Can you work these out from the model? Positions are in its coordinate system, mm. Face numbers are marked on the shaded views. A direction names the side the tool comes from. Round coordinates to 2 decimals unless told otherwise and drop trailing zeros. Order: outer loops, then holes, each group sorted by start corner. A loop starts at its lowest first (then second) coordinate and runs counter-clockwise, first axis right, second up.
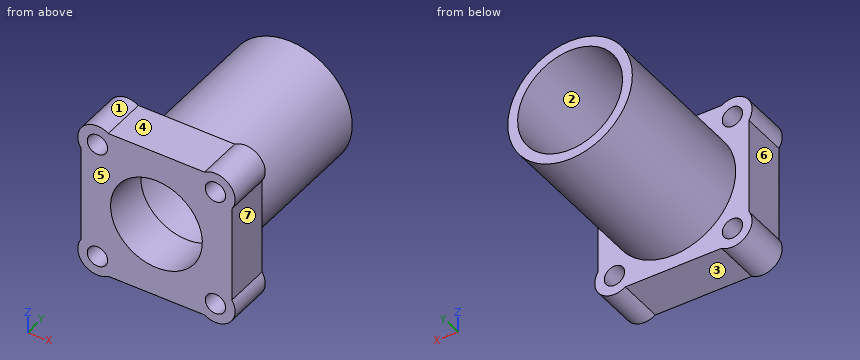
from build123d import *

# Parameters (mm, degrees)
SKETCH_1_R      = 7
SKETCH_1_R_2    = 3
SKETCH_1_R_3    = 1.55
EXTRUDE_1_DEPTH = 7
SKETCH_2_R      = 9.5
SKETCH_2_R_2    = 8
EXTRUDE_2_DEPTH = 24


with BuildPart() as part:
    # 草图1 → 凸台-拉伸1 (new body)
    # profile 1 of 5: a face of its own
    with BuildSketch(Plane(origin=(0, 0, 0), x_dir=(1, 0, 0), z_dir=(0, 1, 0))):
        with BuildLine():
            Line((7.341687605, 11.5), (-7.341687605, 11.5))
            ThreePointArc((-7.341687605, 11.5), (-6.356617963, 10.418637165), (-6, 9))
            ThreePointArc((-6, 9), (-8.133974596, 6.127718677), (-11.5, 7.341687605))
            Line((-11.5, 7.341687605), (-11.5, -7.341687605))
            ThreePointArc((-11.5, -7.341687605), (-8.133974596, -6.127718677), (-6, -9))
            ThreePointArc((-6, -9), (-6.356617963, -10.418637165), (-7.341687605, -11.5))
            Line((-7.341687605, -11.5), (7.341687605, -11.5))
            ThreePointArc((7.341687605, -11.5), (6.878679656, -6.878679656), (11.5, -7.341687605))
            Line((11.5, -7.341687605), (11.5, 7.341687605))
            ThreePointArc((11.5, 7.341687605), (6.878679656, 6.878679656), (7.341687605, 11.5))
        make_face()
        with Locations(Location((0, 0, 0), (0, 0, 270))):
            Circle(SKETCH_1_R, mode=Mode.SUBTRACT)
    # profile 2 of 5: a face of its own
    with BuildSketch(Plane(origin=(0, 0, 0), x_dir=(1, 0, 0), z_dir=(0, 1, 0))):
        with Locations((-9, -9)):
            Circle(SKETCH_1_R_2)
        with Locations(Location((-9, -9, 0), (0, 0, 270))):
            Circle(SKETCH_1_R_3, mode=Mode.SUBTRACT)
    # profile 3 of 5: a face of its own
    with BuildSketch(Plane(origin=(0, 0, 0), x_dir=(1, 0, 0), z_dir=(0, 1, 0))):
        with Locations((9, -9)):
            Circle(SKETCH_1_R_2)
        with Locations(Location((9, -9, 0), (0, 0, 270))):
            Circle(SKETCH_1_R_3, mode=Mode.SUBTRACT)
    # profile 4 of 5: a face of its own
    with BuildSketch(Plane(origin=(0, 0, 0), x_dir=(1, 0, 0), z_dir=(0, 1, 0))):
        with Locations((9, 9)):
            Circle(SKETCH_1_R_2)
        with Locations(Location((9, 9, 0), (0, 0, 270))):
            Circle(SKETCH_1_R_3, mode=Mode.SUBTRACT)
    # profile 5 of 5: a face of its own
    with BuildSketch(Plane(origin=(0, 0, 0), x_dir=(1, 0, 0), z_dir=(0, 1, 0))):
        with Locations((-9, 9)):
            Circle(SKETCH_1_R_2)
        with Locations(Location((-9, 9, 0), (0, 0, 270))):
            Circle(SKETCH_1_R_3, mode=Mode.SUBTRACT)
    extrude(amount=EXTRUDE_1_DEPTH)

    # 草图2 → 凸台-拉伸2 (add)
    with BuildSketch(Plane(origin=(0, 7, 0), x_dir=(1, 0, 0), z_dir=(0, 1, 0))):
        with Locations(Location((0, 0, 0), (0, 0, 270))):
            Circle(SKETCH_2_R)
        with Locations(Location((0, 0, 0), (0, 0, 270))):
            Circle(SKETCH_2_R_2, mode=Mode.SUBTRACT)
    extrude(amount=EXTRUDE_2_DEPTH)


solid = part.part
(1) Please list where these lines run through material, in increasing order: probe 1 along X at (y, z) = (2, -9); probe 2 along X at (y, z) = (26, 0); probe 3 along Z at (x, y) = (1.5, 10).
(2) I'm going to push flat-ended pins straight in: pin 1 Ø4 at (x, z) = (-9, -9) entering from +Y; pin 2 Ø3.5 at (y, z) = (3.5, -2.5) entering from -X; pin 3 Ø4 at (x, y) = (-1.5, 6.5) entering from -Z. Where does each tip first touch, or does it pass through?
(3) I want a section at D-D, the plane x = -9. List the corners of the cut face in (y, z) for me.
(4) On a 3-axis mill with a long thin cutter (end or side, diameter ignored), from which of +Z, -Z, +X, -X, +Y, -Y can I reach the whole of each face in a straight line? I mean the marked faces 1, 2 and 3. Say none if no direction works.
(5) If we mould it in two halves opening along X, with no side actions, what happens to the marked faces 4, 5, 6 and 7? For each: pulls with the +X half, pulls with the -X half, needs draft (parallel to the pull), parting line crosses it, or undercut.
(6) I want a section at B-B, the plane z = 0. List the corners of the cut face in (x, y) for me, plus the area to 3 significant figures.
(7) I want a section at A-A, the plane x = 0. List the corners of the cut face in (y, z) for me, plus the area to 3 significant figures.
(8) I want a section at C-C, the plane z = -9. List the corners of the cut face in (x, y) for me.
Ans:
1. probe 1: x = -12 to -10.55, -7.45 to 7.45, 10.55 to 12
1. probe 2: x = -9.5 to -8, 8 to 9.5
1. probe 3: z = -9.38 to -7.86, 7.86 to 9.38
2. pin 1: stops at y = 7
2. pin 2: stops at x = -11.5
2. pin 3: stops at z = -11.5
3. outline: (0, -12) - (7, -12) - (7, -10.55) - (0, -10.55) - close; (0, -7.45) - (7, -7.45) - (7, -3.04) - (31, -3.04) - (31, 3.04) - (7, 3.04) - (7, 7.45) - (0, 7.45) - close; (0, 10.55) - (7, 10.55) - (7, 12) - (0, 12) - close
4. face 1: +Y, -Y
4. face 2: +Y
4. face 3: -Z, +Y, -Y
5. face 4: undercut
5. face 5: needs draft
5. face 6: pulls with the -X half
5. face 7: pulls with the +X half
6. outline: (-11.5, 0) - (-7, 0) - (-7, 7) - (-8, 7) - (-8, 31) - (-9.5, 31) - (-9.5, 7) - (-11.5, 7) - close; (7, 0) - (11.5, 0) - (11.5, 7) - (9.5, 7) - (9.5, 31) - (8, 31) - (8, 7) - (7, 7) - close
6. area: 135 mm2
7. outline: (0, -11.5) - (7, -11.5) - (7, -9.5) - (31, -9.5) - (31, -8) - (7, -8) - (7, -7) - (0, -7) - close; (0, 7) - (7, 7) - (7, 8) - (31, 8) - (31, 9.5) - (7, 9.5) - (7, 11.5) - (0, 11.5) - close
7. area: 135 mm2
8. outline: (-12, 0) - (-10.55, 0) - (-10.55, 7) - (-12, 7) - close; (-7.45, 0) - (7.45, 0) - (7.45, 7) - (3.04, 7) - (3.04, 31) - (-3.04, 31) - (-3.04, 7) - (-7.45, 7) - close; (10.55, 0) - (12, 0) - (12, 7) - (10.55, 7) - close
